Design review of the part shown in the three views and the two pictorial views. Dimensions are in mm from the part's minimum x, y and z. A direction names the side the tool comes from. Coordinates: 2 decimals unless noted, no trailing zeros. Loops run counter-clockwise (first coordinate to the right, second up) from the corner with the lowest first, then second, coordinate; pieces in that order, holes last. Notation, with made-up numbers: (17, -32.75) -> (33, -32.75) arc R10 ccw to (33, -21.75) -> close; hole circle Ø3 at (10, -5). An arc over 180 degrees is marked (long way). One line per item, written item: value. Start each with the question number.
1. For probe 1 along X at (y, z) = (2.25, 20) (1 decimal); probe 2 along X at (y, z) = (84.55, 20) (1 decimal); probe 3 along Y at (x, z) = (143.5, 22.5), list the stretches that pass through material, from the lowest coordinate up.
2. Add section C-C on z = 8. Write out the cut boundary in (x, y) (1 decimal), plus the area to 3 significant figures.
3. Add section A-A on x = 58.5. Write out the cut boundary in (y, z), plus the area to 3 significant figures.
4. Machinability: for the marked faces 4, 5 and 6, which of the approach directions +Z, -Z, +X, -X, +Y, -Y give a long, thin tool a straight path to every point of the face, cutting with its end or side? Answer none if there is none.
5. Add section D-D on y = 53. Write out the cut boundary in (x, z) (1 decimal), plus the area to 3 significant figures.
6. Add section B-B on z = 20. Give the number of separate pieces and of enclosed holes in the cut face, plus the area to 3 significant figures.
7. Draft analysis for pull direction Y (two halves, no side actions). For the marked faces 1, 2 and 3, state which applies: pulls with the +Y half, pulls with the -Y half, needs draft (parallel to the pull), parting line crosses it, or undercut.
8. Insertion check: pin 1 (10 mm diameter, centred on x = 76, z = 31.5, fed in from +Y); pin 2 (5 mm diameter, centred on x = 154, y = 63, fed in from +Z); pin 3 (6 mm diameter, centred on x = 140, z = 20.5, fed in from -Y); pin 4 (7 mm diameter, centred on x = 138.4, z = 20, fed in from +Y). Each pin has a flat end and moves straight along its axis. Give the tip position at first contact, or say it passes through.
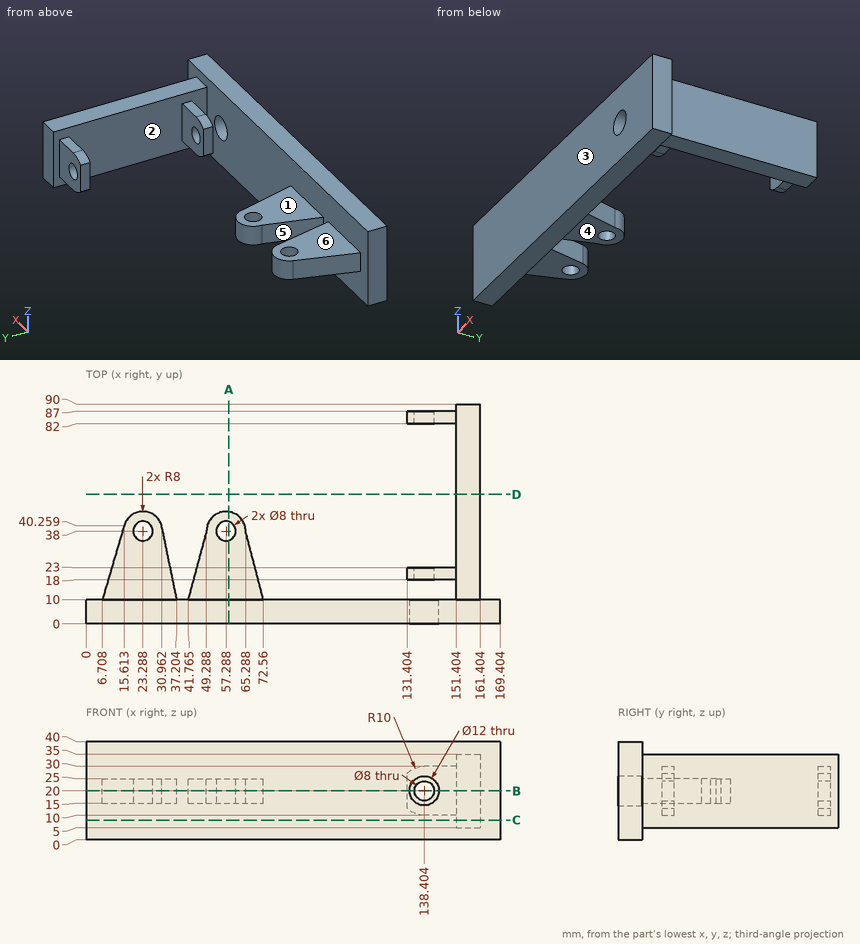
Worked answers:
1. probe 1: x = 0 to 132.4, 144.4 to 169.4
1. probe 2: x = 131.4 to 134.4, 142.4 to 161.4
1. probe 3: y = 18 to 23, 82 to 87
2. outline: (0, 0) -> (169.4, 0) -> (169.4, 10) -> (161.4, 10) -> (161.4, 90) -> (151.4, 90) -> (151.4, 10) -> (0, 10) -> close
2. area: 2,490 mm²
3. outline: (0, 0) -> (10, 0) -> (10, 15) -> (34.19, 15) -> (34.19, 25) -> (10, 25) -> (10, 40) -> (0, 40) -> close; (41.81, 15) -> (45.91, 15) -> (45.91, 25) -> (41.81, 25) -> close
3. area: 683 mm²
4. face 4: -Z, -X, +Y
4. face 5: +Z, -Z, +Y
4. face 6: +Z, -X, +Y
5. outline: (151.4, 5) -> (161.4, 5) -> (161.4, 35) -> (151.4, 35) -> close
5. area: 300 mm²
6. separate pieces: 4
6. enclosed holes: 2
6. area: 3,910 mm²
7. face 1: needs draft
7. face 2: undercut
7. face 3: pulls with the -Y half
8. pin 1: stops at y = 10
8. pin 2: stops at z = 35
8. pin 3: stops at y = 18
8. pin 4: passes through
